```python
from build123d import *

# Parameters (mm, degrees)
SKETCH1_W             = 48
SKETCH1_H             = 36
SKETCH1_R             = 7.5
BOSS_EXTRUDE1_DEPTH   = 25
SKETCH2_R             = 12
CUT_EXTRUDE1_DEPTH    = 5
SKETCH3_R             = 9.9
CUT_EXTRUDE2_DEPTH    = 3
SKETCH5_R             = 2
CUT_EXTRUDE3_DEPTH    = 20
M5_TAPPED_HOLE1_D     = 4.2
M5_TAPPED_HOLE1_DEPTH = 12.4
M5_TAPPED_HOLE1_TIP   = 1.2618073
M3_TAPPED_HOLE1_D     = 2.5
M3_TAPPED_HOLE1_DEPTH = 10.1
M3_TAPPED_HOLE1_TIP   = 0.751075774


with BuildPart() as part:
    # Sketch1 → Boss-Extrude1 (new, symmetric)
    with BuildSketch(Plane(origin=(0, 0, 0), x_dir=(0, 0, -1), z_dir=(1, 0, 0))):
        Rectangle(SKETCH1_W, SKETCH1_H)
        Circle(SKETCH1_R, mode=Mode.SUBTRACT)
    extrude(amount=BOSS_EXTRUDE1_DEPTH, both=True)

    # Sketch2 → Cut-Extrude1 (cut)
    with BuildSketch(Plane.ZY.offset(25)):
        Circle(SKETCH2_R)
    cut_extrude1 = extrude(amount=-CUT_EXTRUDE1_DEPTH, mode=Mode.SUBTRACT)

    # Sketch3 → Cut-Extrude2 (cut)
    with BuildSketch(Plane.ZY.offset(20)):
        Circle(SKETCH3_R)
    cut_extrude2 = extrude(amount=-CUT_EXTRUDE2_DEPTH, mode=Mode.SUBTRACT)

    # Mirror4: Cut-Extrude1, Cut-Extrude2 across plane
    add(cut_extrude1.mirror(Plane(origin=(0, 0, 0), x_dir=(0, 0, 1), z_dir=(1, 0, 0))), mode=Mode.SUBTRACT)
    add(cut_extrude2.mirror(Plane(origin=(0, 0, 0), x_dir=(0, 0, 1), z_dir=(1, 0, 0))), mode=Mode.SUBTRACT)

    # Sketch5 → Cut-Extrude3 (cut)
    with BuildSketch(Plane(origin=(0, 0, -24), x_dir=(-1, 0, 0), z_dir=(0, 0, -1))):
        with Locations((7, 0)):
            Circle(SKETCH5_R)
        with Locations((-7, 0)):
            Circle(SKETCH5_R)
    extrude(amount=-CUT_EXTRUDE3_DEPTH, mode=Mode.SUBTRACT)

    # M5 Tapped Hole1
    with Locations(Plane(origin=(25, 0, 0), x_dir=(0, 0, -1), z_dir=(1, 0, 0))):
        with Locations((-18, 14), (18, 14), (-18, -14), (18, -14)):
            Hole(M5_TAPPED_HOLE1_D / 2, depth=M5_TAPPED_HOLE1_DEPTH)
            with Locations((0, 0, -(M5_TAPPED_HOLE1_DEPTH + M5_TAPPED_HOLE1_TIP / 2))):  # 118° drill point
                Cone(0, M5_TAPPED_HOLE1_D / 2, M5_TAPPED_HOLE1_TIP, mode=Mode.SUBTRACT)

    # M3 Tapped Hole1
    with Locations(Plane.ZY.offset(25)):
        with Locations((-14, 14), (-14, -14), (14, 14), (14, -14)):
            Hole(M3_TAPPED_HOLE1_D / 2, depth=M3_TAPPED_HOLE1_DEPTH)
            with Locations((0, 0, -(M3_TAPPED_HOLE1_DEPTH + M3_TAPPED_HOLE1_TIP / 2))):  # 118° drill point
                Cone(0, M3_TAPPED_HOLE1_D / 2, M3_TAPPED_HOLE1_TIP, mode=Mode.SUBTRACT)


solid = part.part
```
Read the model definition and answer for the solid it produces. Units are mm, in the model's axes. A direction names the side the tool comes from. Coordinates: 2 decimals unless noted, no trailing zeros. Write each loop counter-clockwise with the first axis right and the second up, starting at its lowest first coordinate (ties: lowest second). Pieces come first, ordered by that corner, then holes. Notation, with made-up numbers: (21.5, 31) - (26.5, 31) arc R21 ccw to (26.5, 50) - close; hole circle Ø4 at (18.5, -33). An arc over 180 degrees is marked (long way). Answer as a JSON object with one key per item and string values. Group by question number.
1. A cutting plane is placed at C-C (x = 15). Determine the outline of the cut face in (y, z), plus the area to 3 significant figures.
2. Which of the six approach directions +Z, -Z, +X, -X, +Y, -Y give full straight-line access (tool end or side, diameter ignored) to faces 5 (the cylindrical face through (18.713, 14.631, 20.003)), 6 (the flat face through (0, 0, -24)), 7 (the flat face through (-20, 10, 2))?
3. Each of these flat-tipped pins is pushed along its axis until it touches: P1, Ø18, axis at y = 0, z = 0, coming from the -X side; P2, Ø21.5, axis at y = 0, z = 0, coming from the +X side; P3, Ø12, axis at y = 2, z = 2.5, coming from the +X side. Where does it stop, or does it pass through?
4. A cutting plane is placed at D-D (x = 7). Determine the outline of the cut face in (y, z).
5. A cutting plane is placed at A-A (y = 4). Determine the outline of the cut face in (x, z).
6. A cutting plane is placed at B-B (z = 0). Determine the outline of the cut face in (x, y).
7. The mould has two halves that part along Y. Classify faces 1 (the cylindrical face through (-22.54, 0.53, -11.99)), 2 (the flat face through (0, 0, 24)), 3 (the cylindrical face through (-5, 0, -16)), 4 (the flat face through (0, 18, 0)): +Y half, -Y half, draft (parallel to the pull), parting line (faces both ways), or undercut.
8. Consider L1, parallel to Z at x = 19, y = 14; L2, parallel to Y at x = 20, z = -18; L3, parallel to Y at x = -18.25, z = 14. Determine where each line is inside the solid, lowest interval first. Write a range as [from, to].
Worked out:
{
 "1": {"outline": "(-18, -24) - (18, -24) - (18, 24) - (-18, 24) - close; hole circle Ø4.2 at (-14, -18); hole circle Ø4.2 at (-14, 18); hole circle Ø15 at (0, 0); hole circle Ø4.2 at (14, -18); hole circle Ø4.2 at (14, 18)", "area": "1,500 mm²"},
 "2": {"face 5": "+X", "face 6": "-Z, +X, -X, +Y, -Y", "face 7": "-X"},
 "3": {"P1": "stops at x = -17", "P2": "stops at x = 20", "P3": "stops at x = 17"},
 "4": {"outline": "(-18, -24) - (-2, -24) - (-2, -7.23) arc R7.5 cw (long way) to (2, -7.23) - (2, -24) - (18, -24) - (18, 24) - (-18, 24) - close"},
 "5": {"outline": "(-25, -24) - (25, -24) - (25, -11.31) - (20, -11.31) - (20, -9.06) - (17, -9.06) - (17, -6.34) - (-17, -6.34) - (-17, -9.06) - (-20, -9.06) - (-20, -11.31) - (-25, -11.31) - close; (-25, 11.31) - (-20, 11.31) - (-20, 9.06) - (-17, 9.06) - (-17, 6.34) - (17, 6.34) - (17, 9.06) - (20, 9.06) - (20, 11.31) - (25, 11.31) - (25, 24) - (-25, 24) - close"},
 "6": {"outline": "(-25, -18) - (25, -18) - (25, -12) - (20, -12) - (20, -9.9) - (17, -9.9) - (17, -7.5) - (-17, -7.5) - (-17, -9.9) - (-20, -9.9) - (-20, -12) - (-25, -12) - close; (-25, 12) - (-20, 12) - (-20, 9.9) - (-17, 9.9) - (-17, 7.5) - (17, 7.5) - (17, 9.9) - (20, 9.9) - (20, 12) - (25, 12) - (25, 18) - (-25, 18) - close"},
 "7": {"face 1": "undercut", "face 2": "draft", "face 3": "undercut", "face 4": "+Y half"},
 "8": {"L1": "z = [-24, -20.1], [-15.9, 15.9], [20.1, 24]", "L2": "y = [-18, -16.1], [-11.9, 11.9], [16.1, 18]", "L3": "y = [-18, -15.25], [-12.75, 12.75], [15.25, 18]"}
}
